Could you check a few things on this model? Use its own coordinates, in mm. A direction names the side the tool comes from. Give positions to 0.01 mm unless a question says otherwise; leave off trailing zeros. Order: outer loops, then holes, each group sorted by start corner. A loop starts at its lowest first (then second) coordinate and runs counter-clockwise, first axis right, second up. Notation, with made-up numbers: (-40, 21.25) - (-19, 21.25) arc R15 cw to (-19, 29.25) - close; hole circle Ø11 at (-17, 57.25). An arc over 180 degrees is marked (long way). Put each result on its own line as item: value.
from build123d import *

# Parameters (mm, degrees)
SKETCH_1_R          = 7.5
EXTRUDE_1_DEPTH     = 158.5
SKETCH_5_OUTSIDE_W  = 48.982
SKETCH_5_OUTSIDE_H  = 48.982
SKETCH_5_OUTSIDE_R  = 6
CUT_EXTRUDE_3_DEPTH = 29.5
CHAMFER_2_SIZE      = 0.5
SKETCH_2_OUTSIDE_W  = 48.982
SKETCH_2_OUTSIDE_H  = 48.982
SKETCH_2_OUTSIDE_R  = 6
CUT_EXTRUDE_4_DEPTH = 10
CHAMFER_3_SIZE      = 0.5
CUT_EXTRUDE_START   = -4
CUT_EXTRUDE_5_DEPTH = 48


with BuildPart() as part:
    # 草图1 → 凸台-拉伸1 (new body)
    with BuildSketch(Plane.XY):
        Circle(SKETCH_1_R)
    extrude(amount=-EXTRUDE_1_DEPTH)

    # 草图5 outside → 切除-拉伸3 (cut)
    with BuildSketch(Plane.XY):
        Rectangle(SKETCH_5_OUTSIDE_W, SKETCH_5_OUTSIDE_H)
        Circle(SKETCH_5_OUTSIDE_R, mode=Mode.SUBTRACT)
    extrude(amount=-CUT_EXTRUDE_3_DEPTH, mode=Mode.SUBTRACT)

    # 倒角2
    chamfer_2_edges = [part.edges().sort_by_distance(p)[0] for p in [
        (-7.5, 0, -29.5),
        (-6, 0, 0),
    ]]
    chamfer(chamfer_2_edges, length=CHAMFER_2_SIZE)

    # 草图2 outside → 切除-拉伸4 (cut)
    with BuildSketch(Plane(origin=(0, 0, -158.5), x_dir=(-1, 0, 0), z_dir=(0, 0, -1))):
        Rectangle(SKETCH_2_OUTSIDE_W, SKETCH_2_OUTSIDE_H)
        with Locations(Location((0, 0, 0), (0, 0, 180))):
            Circle(SKETCH_2_OUTSIDE_R, mode=Mode.SUBTRACT)
    extrude(amount=-CUT_EXTRUDE_4_DEPTH, mode=Mode.SUBTRACT)

    # 倒角3
    chamfer_3_edges = [part.edges().sort_by_distance(p)[0] for p in [
        (-7.5, 0, -148.5),
        (-6, 0, -158.5),
    ]]
    chamfer(chamfer_3_edges, length=CHAMFER_3_SIZE)

    # 草图8 → 切除-拉伸5 (cut)
    with BuildSketch(Plane(origin=(0, 0, 0), x_dir=(1, 0, 0), z_dir=(0, 1, 0)).offset(CUT_EXTRUDE_START)):
        with BuildLine():
            Line((2.5, 57.5), (2.5, 32.5))
            ThreePointArc((2.5, 32.5), (0, 30), (-2.5, 32.5))
            Line((-2.5, 32.5), (-2.5, 57.5))
            ThreePointArc((-2.5, 57.5), (0, 60), (2.5, 57.5))
        make_face()
        with BuildLine():
            Line((2.5, 145.5), (2.5, 120.5))
            ThreePointArc((2.5, 120.5), (0, 118), (-2.5, 120.5))
            Line((-2.5, 120.5), (-2.5, 145.5))
            ThreePointArc((-2.5, 145.5), (0, 148), (2.5, 145.5))
        make_face()
    extrude(amount=-CUT_EXTRUDE_5_DEPTH, mode=Mode.SUBTRACT)


solid = part.part
1) If I drill on line 1 (X direction, y = -2.75, z = -48.5); line 2 (Z direction, x = -4.5, y = -5.25), over which ranges is the centre line in solid material (lowest first)? Write a range as [from, to].
Filled in:
line 1: x = [-6.98, 6.98]
line 2: z = [-148.5, -29.5]
2) Suppose I cut it at A-A, the plane z = -141.5. List the corners of the cut face in (x, y) for me, and give its area (3 significant figures).
Filled in:
outline: (-2.5, -7.07) - (-2.5, -4) - (2.5, -4) - (2.5, -7.07) arc R7.5 ccw (long way) to start
area: 160 mm^2
3) I'm going to push flat-ended pins straight in: pin 1 (3 mm diameter, centred on x = -3.5, z = -47, fed in from +Y); pin 2 (4 mm diameter, centred on x = 1.5, y = -1, fed in from +Z); pin 3 (4 mm diameter, centred on y = -5.5, z = -77, fed in from +X); pin 4 (1.5 mm diameter, centred on y = -5, z = -47, fed in from +X). Where does each tip first touch, or does it pass through?
Filled in:
pin 1: stops at y = 7.23
pin 2: stops at z = 0
pin 3: stops at x = 6.63
pin 4: stops at x = 6.18
4) Which directions (+Z, -Z, +X, -X, +Y, -Y) give clear straight access to the entire face, cutting with the end or side of a thin tool? Please do faces 4 (the flat face through (-6, 2, -148.5)), 5 (the flat face through (6, 2, -29.5)), 6 (the flat face through (0, 0, -158.5)), 7 (the flat face through (2.5, -6, -45)).
Filled in:
face 4: -Z
face 5: +Z
face 6: -Z, +X, -X, +Y, -Y
face 7: -Y
5) We'd pull the mould along Z, two halves only. Please class faces 1 (the flat face through (0, 0, 0)), 2 (the flat face through (-2.5, -6, -133)), 3 (the cylindrical face through (5.723, -1.802, -153.316)): pulls with the +Z half, pulls with the -Z half, needs draft (parallel to the pull), parting line crosses it, or undercut.
Filled in:
face 1: pulls with the +Z half
face 2: undercut
face 3: needs draft
